Check sheet for the modelled part. Datum: model origin and axes. Units: mm. A direction names the side the tool comes from. Coordinates: 2 decimals unless noted, no trailing zeros. Loops run counter-clockwise (first coordinate to the right, second up) from the corner with the lowest first, then second, coordinate; pieces in that order, holes last. Notation, with made-up numbers: (-29, 86) - (-22, 86) arc R26 ccw to (-22, 125) - close; hole circle Ø3 at (88, -8). An arc over 180 degrees is marked (long way). Write each question's results on one line, items separated by ' | '. Start each with the question number.
1. Cross-section at A-A (z = 0). Record the cut outline in (x, y).
2. Cross-section at C-C (y = -135.5). Record the cut outline in (x, z).
3. Draft check along Y on faces 1 (the face through (2, -660, 2)), 2 (the face through (34.471, -295.8, 83.137)), 3 (the face through (41.3, 22.18, 131.15)). Enter one of: released by +Y, released by -Y, zero draft, split by the parting line, or undercut.
4. Thickness scan on line 1 (Y direction, x = 83.5, z = -82.5); line 2 (Y direction, x = 139, z = 48); line 3 (Z direction, x = -5, y = -484). Record the ranges inside material, lowest first. Write a range as [from, to].
5. Gauge pin test, flat ends, axial feed: P1, Ø2, axis at y = -60.5, z = 17.5, coming from the +X side; P2, Ø8, axis at x = 0, y = -223, coming from the -Z side; P3, Ø10, axis at y = -255, z = 48.5, coming from the +X side. Record the tip position at first contact, or that the pin passes through.
6. Tool access check on faces 4 (the face through (-64, -600, -64)), 5 (the face through (156.836, -634.65, 20.592)). Record the directions out of +Z, -Z, +X, -X, +Y, -Y that give a thin tool (end or side, any length) a straight path to the whole face; none if there is none.
7. Cross-section at B-B (x = 0). Record the cut outline in (y, z).
```python
from build123d import *

# Parameters (mm, degrees)
SKETCH1_R           = 137.5
BOSS_EXTRUDE1_DEPTH = 45
SKETCH2_R           = 90
BOSS_EXTRUDE2_DEPTH = 600
SKETCH3_R           = 158.18220737
BOSS_EXTRUDE3_DEPTH = 60
FILLET1_R           = 10


with BuildPart() as part:
    # Sketch1 → Boss-Extrude1 (new body)
    with BuildSketch(Plane(origin=(0, 0, 0), x_dir=(1, 0, 0), z_dir=(0, 1, 0))):
        with Locations(Location((0, 0, 0), (0, 0, 270))):
            Circle(SKETCH1_R)
    extrude(amount=BOSS_EXTRUDE1_DEPTH)

    # Sketch2 → Boss-Extrude2 (add)
    with BuildSketch(Plane.XZ):
        with Locations(Location((0, 0, 0), (0, 0, 90))):
            Circle(SKETCH2_R)
    extrude(amount=BOSS_EXTRUDE2_DEPTH)

    # Sketch3 → Boss-Extrude3 (add)
    with BuildSketch(Plane.XZ.offset(600)):
        with Locations(Location((0, 0, 0), (0, 0, 270))):
            Circle(SKETCH3_R)
    extrude(amount=BOSS_EXTRUDE3_DEPTH)

    # Fillet1
    fillet1_edges = [part.edges().sort_by_distance(p)[0] for p in [
        (0, -600, 158.18220737),
    ]]
    fillet(fillet1_edges, radius=FILLET1_R)


solid = part.part
```
Established:
1) outline: (-158.18, -660) - (158.18, -660) - (158.18, -610) arc R10 ccw to (148.18, -600) - (90, -600) - (90, 0) - (137.5, 0) - (137.5, 45) - (-137.5, 45) - (-137.5, 0) - (-90, 0) - (-90, -600) - (-148.18, -600) arc R10 ccw to (-158.18, -610) - close
2) outline: circle Ø180 at (0, 0)
3) face 1: released by -Y | face 2: undercut | face 3: zero draft
4) line 1: [-660, -600], [0, 45] | line 2: [-660, -600] | line 3: [-89.86, 89.86]
5) P1: x = 88.47 | P2: z = -90 | P3: x = 78.79
6) face 4: none | face 5: +Y, -Y
7) outline: (-660, -158.18) - (-610, -158.18) arc R10 ccw to (-600, -148.18) - (-600, -90) - (0, -90) - (0, -137.5) - (45, -137.5) - (45, 137.5) - (0, 137.5) - (0, 90) - (-600, 90) - (-600, 148.18) arc R10 ccw to (-610, 158.18) - (-660, 158.18) - close
